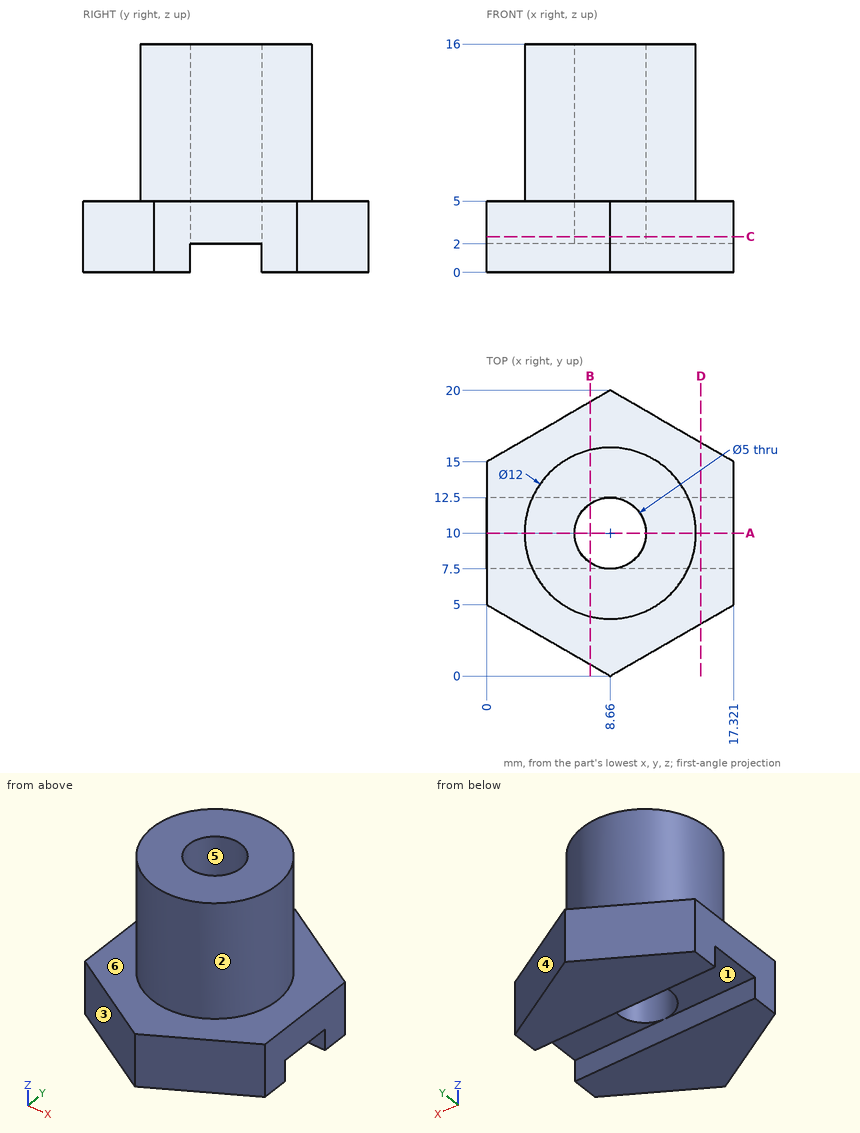
Here's the drawing with two shaded views (mm, measured from the low corner). I have some questions. A direction names the side the tool comes from. Round coordinates to 2 decimals unless told otherwise and drop trailing zeros. Loops run counter-clockwise (first coordinate to the right, second up) from the corner with the lowest first, then second, coordinate; pieces in that order, holes last.
Item 1: If we mould it in two halves opening along X, with no side actions, what happens to the marked faces 4, 5 and 6? For each: +X half, -X half, draft (parallel to the pull), parting line (faces both ways), or undercut.
Item 2: Will these pins go through, and if not, where does the flat tip stop? pin 1 Ø4 at (x, z) = (12, 9.5) entering from -Y; pin 2 Ø2 at (x, z) = (12, 1) entering from -Y; pin 3 Ø1 at (x, z) = (14, 11) entering from +Y (1 decimal).
Item 3: Suppose I cut it at A-A, the plane y = 10. Write out the boundary of the cut face in (x, z), then the cut area to 3 significant figures.
Item 4: Which directions (+Z, -Z, +X, -X, +Y, -Y) give clear straight access to the entire face, cutting with the end or side of a thin tool? Please do the marked faces 1, 2 and 3.
Item 5: Suppose I cut it at C-C, the plane z = 2.5. Write out the boundary of the cut face in (x, y), then the cut area to 3 significant figures.
Item 6: Please list where these lines run through material, in increasing order: L1, parallel to X at y = 10.25, z = 11.5 (1 decimal); L2, parallel to Z at x = 3.25, y = 7.25; L3, parallel to Y at x = 6.5, z = 8.5 (1 decimal).
Item 7: Suppose I cut it at B-B, the plane x = 7.25. Write out the boundary of the cut face in (y, z) (1 decimal).
Item 8: Suppose I cut it at D-D, the plane x = 15. Write out the boundary of the cut face in (y, z), then the cut area to 3 significant figures.
Reported:
1. face 4: +X half
1. face 5: undercut
1. face 6: draft
2. pin 1: stops at y = 4.15
2. pin 2: stops at y = 1.35
2. pin 3: stops at y = 13.5
3. outline: (0, 2) - (6.16, 2) - (6.16, 16) - (2.66, 16) - (2.66, 5) - (0, 5) - close; (11.16, 2) - (17.32, 2) - (17.32, 5) - (14.66, 5) - (14.66, 16) - (11.16, 16) - close
3. area: 114 mm2
4. face 1: -Z, +X, -X
4. face 2: +Z
4. face 3: +Z, -Z, -X, -Y
5. outline: (0, 5) - (8.66, 0) - (17.32, 5) - (17.32, 15) - (8.66, 20) - (0, 15) - close; hole circle Ø5 at (8.66, 10)
5. area: 240 mm2
6. L1: x = 2.7 to 6.2, 11.1 to 14.7
6. L2: z = 0 to 5
6. L3: y = 4.4 to 8.7, 11.3 to 15.6
7. outline: (0.8, 0) - (7.5, 0) - (7.5, 2) - (7.9, 2) - (7.9, 16) - (4.2, 16) - (4.2, 5) - (0.8, 5) - close; (12.1, 2) - (12.5, 2) - (12.5, 0) - (19.2, 0) - (19.2, 5) - (15.8, 5) - (15.8, 16) - (12.1, 16) - close
8. outline: (3.66, 0) - (7.5, 0) - (7.5, 2) - (12.5, 2) - (12.5, 0) - (16.34, 0) - (16.34, 5) - (3.66, 5) - close
8. area: 53.4 mm2
